```python
from build123d import *

# Parameters (mm, degrees)
ARM_PROFILE_SKETCH_R  = 0.95
ARM_BODY_DEPTH        = 2.625
FORK_SLOT_SKETCH_W    = 39.128483504
FORK_SLOT_SKETCH_H    = 2.75
FORK_SLOT_CUT_DEPTH   = 22.625
CENTRE_WEB_DEPTH      = 2.625
CENTRE_WEB_DEPTH_BACK = 1.375


with BuildPart() as part:
    # Arm Profile Sketch → Arm Body (new, symmetric)
    with BuildSketch(Plane(origin=(0, 0, 0), x_dir=(1, 0, 0), z_dir=(0, 1, 0))):
        with BuildLine():
            Line((-17.15759803, 1.993781046), (-0.196997537, 3.334428369))
            ThreePointArc((-0.196997537, 3.334428369), (0, 3.342202061), (0.196997537, 3.334428369))
            Line((0.196997537, 3.334428369), (17.15759803, 1.993781046))
            ThreePointArc((17.15759803, 1.993781046), (18.998552025, 0.076090769), (17.308740296, -1.976026171))
            Line((17.308740296, -1.976026171), (0.386342216, -4.620032749))
            ThreePointArc((0.386342216, -4.620032749), (0, -4.65), (-0.386332201, -4.619903915))
            Line((-0.386332201, -4.619903915), (-17.15759803, -1.993781046))
            ThreePointArc((-17.15759803, -1.993781046), (-19, 0), (-17.15759803, 1.993781046))
        make_face()
        with Locations(Location((-17, 0, 0), (0, 0, 90))):
            Circle(ARM_PROFILE_SKETCH_R, mode=Mode.SUBTRACT)
        with Locations(Location((17, 0, 0), (0, 0, 90))):
            Circle(ARM_PROFILE_SKETCH_R, mode=Mode.SUBTRACT)
        with Locations(Location((0, -1.75, 0), (0, 0, 90))):
            Circle(ARM_PROFILE_SKETCH_R, mode=Mode.SUBTRACT)
    extrude(amount=ARM_BODY_DEPTH, both=True)

    # Fork Slot Sketch → Fork Slot Cut (cut, symmetric)
    with BuildSketch(Plane.XY):
        Rectangle(FORK_SLOT_SKETCH_W, FORK_SLOT_SKETCH_H)
    extrude(amount=FORK_SLOT_CUT_DEPTH, both=True, mode=Mode.SUBTRACT)


with BuildPart() as fork_slot_cut_piece_1:
    # of the separate pieces the step leaves, piece 1, a body of its own (fork_slot_cut_pieces)
    add(part.part.solids().sort_by_distance((-0.386332201, -2.625, 4.619903915))[0])



with BuildPart() as fork_slot_cut_piece_2:
    # of the separate pieces the step leaves, piece 2, a body of its own (fork_slot_cut_pieces)
    add(part.part.solids().sort_by_distance((-0.386332201, 1.375, 4.619903915))[0])


with BuildPart() as fork_slot_cut_piece_1_1:
    add(fork_slot_cut_piece_1.part)

    add(fork_slot_cut_piece_2.part)  # Centre Web merges Fork Slot Cut piece 2
    # Centre Web Sketch → Centre Web (add, two sides: drawn at the far end of the back side and taken through both)
    with BuildSketch(Plane(origin=(0, 0, 0), x_dir=(1, 0, 0), z_dir=(0, 1, 0)).offset(-CENTRE_WEB_DEPTH_BACK)):
        with BuildLine():
            Line((6.720689655, -1.718976713), (11.853914762, 0.981023287))
            ThreePointArc((11.853914762, 0.981023287), (12.664248394, 0.729310345), (12.412535452, -0.081023287))
            Line((12.412535452, -0.081023287), (7.279310345, -2.781023287))
            ThreePointArc((7.279310345, -2.781023287), (6.468976713, -2.529310345), (6.720689655, -1.718976713))
        make_face()
    extrude(amount=CENTRE_WEB_DEPTH + CENTRE_WEB_DEPTH_BACK)


solid = fork_slot_cut_piece_1_1.part
```
Source: CAD feature listing. Evaluate the final solid. Frame: model axes, mm. A direction names the side the tool comes from. Round coordinates to 2 decimals unless told otherwise and drop trailing zeros. Order: outer loops, then holes, each group sorted by start corner. A loop starts at its lowest first (then second) coordinate and runs counter-clockwise, first axis right, second up. Notation, with made-up numbers: (39, -23.75) -> (70, -23.75) arc R18 cw to (70, -1.75) -> close; hole circle Ø9 at (2.5, -23.75). An arc over 180 degrees is marked (long way). Use CSV: the item, a comma, the result in double quotes.
(1) Pull-direction query (Y, two-part tool) for faces 1 (the face through (0.3, -2.625, 0.6)), 2 (the face through (12.66, -0.02, -0.74)), 3 (the face through (17.84, -2.01, -0.44)); classes: +Y half, -Y half, draft (parallel to the pull), parting line (faces both ways), or undercut.
Report:
face 1,"-Y half"
face 2,"undercut"
face 3,"draft"
(2) First-contact query: pin 1 Ø1.5 at (y, z) = (-2, 1.5) entering from +X. Flat tip, straight axial feed; report the tip coordinate or a pass-through.
Report:
pin 1,"x = 18.85"
(3) Section D-D on y = -0.1. Return the cut outline in (x, z), and give its area (3 significant figures).
Report:
outline,"(6.72, 1.72) -> (11.85, -0.98) arc R0.6 ccw to (12.41, 0.08) -> (7.28, 2.78) arc R0.6 ccw to start"
area,"8.09 mm^2"
(4) Section C-C on x = 15.5. Return the cut outline in (y, z) (3 decimals).
Report:
outline,"(-2.625, -2.125) -> (-1.375, -2.125) -> (-1.375, 2.259) -> (-2.625, 2.259) -> close; (1.375, -2.125) -> (2.625, -2.125) -> (2.625, 2.259) -> (1.375, 2.259) -> close"
(5) Ray query, L1, parallel to X at y = -1.75, z = 0; L2, parallel to Y at x = -13.5, z = 1 (3 decimals); L3, parallel to X at y = 1.75, z = -0.75. Return the intervals inside material, ascending.
Report:
L1,"-19 to -17.95, -16.05 to 16.05, 17.95 to 19"
L2,"-2.625 to -1.375, 1.375 to 2.625"
L3,"-18.85 to -17.58, -16.42 to 16.42, 17.58 to 18.85"
(6) Access query for faces 4 (the face through (9.25, -0.02, 0.39)), 5 (the face through (9.882, -0.019, 1.412)), 6 (the face through (17.84, 1.99, -0.44)). Directions: +Z, -Z, +X, -X, +Y, -Y. A direction counts if a zero-diameter tool reaches every point of the face in a straight line with its end or side. Return the directions, or none.
Report:
face 4,"-Z, -X"
face 5,"+Z, +X"
face 6,"+Y, -Y"
(7) Section B-B on z = -3. Return the cut outline in (x, y) (3 decimals).
Report:
outline,"(-4.428, -2.625) -> (4.428, -2.625) -> (4.428, -1.375) -> (-4.428, -1.375) -> close; (-4.428, 1.375) -> (4.428, 1.375) -> (4.428, 2.625) -> (-4.428, 2.625) -> close"
(8) Section A-A on y = 1.9. Return the cut outline in (x, z).
Report:
outline,"(-17.16, -1.99) -> (-0.2, -3.33) arc R2.5 ccw to (0.2, -3.33) -> (17.16, -1.99) arc R2 ccw to (17.31, 1.98) -> (0.39, 4.62) arc R2.5 ccw to (-0.39, 4.62) -> (-17.16, 1.99) arc R2 ccw to start; hole circle Ø1.9 at (-17, 0); hole circle Ø1.9 at (0, 1.75); hole circle Ø1.9 at (17, 0)"
